The model under review builds one solid part; all positions refer to its coordinate system, in mm. A direction names the side the tool comes from. Coordinates: 2 decimals unless noted, no trailing zeros. Write each loop counter-clockwise with the first axis right and the second up, starting at its lowest first coordinate (ties: lowest second). Pieces come first, ordered by that corner, then holes. Notation, with made-up numbers: M 52,17.5 L 100,17.5 A26 cw 100,38.5 Z; hole C 49.25,11.25 d1. An arc over 180 degrees is marked long. Answer as CSV lines item,"result". Start each with the question number.
from build123d import *

# Parameters (mm, degrees)
EXTRUDE_1_DEPTH     = 40
CHAMFER_1_SIZE      = 3
CUT_EXTRUDE_1_DEPTH = 40
SKETCH_4_R          = 2.25
CUT_EXTRUDE_2_DEPTH = 40


with BuildPart() as part:
    # 草图2 → 凸台-拉伸1 (new body)
    with BuildSketch(Plane.XY):
        with BuildLine():
            Line((0, 0), (14.5, 0))
            ThreePointArc((14.5, 0), (16.621320344, 0.878679656), (17.5, 3))
            Line((17.5, 3), (17.5, 8))
            ThreePointArc((17.5, 8), (18.964466094, 11.535533906), (22.5, 13))
            Line((22.5, 13), (67.5, 13))
            ThreePointArc((67.5, 13), (71.035533906, 11.535533906), (72.5, 8))
            Line((72.5, 8), (72.5, 3))
            ThreePointArc((72.5, 3), (73.378679656, 0.878679656), (75.5, 0))
            Line((75.5, 0), (90, 0))
            Line((90, 0), (90, -2))
            Line((90, -2), (75.5, -2))
            ThreePointArc((75.5, -2), (71.964466094, -0.535533906), (70.5, 3))
            Line((70.5, 3), (70.5, 8))
            ThreePointArc((70.5, 8), (69.621320344, 10.121320344), (67.5, 11))
            Line((67.5, 11), (22.5, 11))
            ThreePointArc((22.5, 11), (20.378679656, 10.121320344), (19.5, 8))
            Line((19.5, 8), (19.5, 3))
            ThreePointArc((19.5, 3), (18.035533906, -0.535533906), (14.5, -2))
            Line((14.5, -2), (0, -2))
            Line((0, -2), (0, 0))
        make_face()
    extrude(amount=EXTRUDE_1_DEPTH)

    # 倒角1
    chamfer_1_edges = [part.edges().sort_by_distance(p)[0] for p in [
        (0, -1, 0),
        (90, -1, 0),
        (0, -1, 40),
        (90, -1, 40),
    ]]
    chamfer(chamfer_1_edges, length=CHAMFER_1_SIZE)

    # 草图3 → 切除-拉伸1 (cut)
    with BuildSketch(Plane(origin=(0, 0, 0), x_dir=(1, 0, 0), z_dir=(0, 1, 0))):
        with BuildLine():
            Line((4.25, -10), (4.25, -30))
            ThreePointArc((4.25, -30), (7.5, -33.25), (10.75, -30))
            Line((10.75, -30), (10.75, -10))
            ThreePointArc((10.75, -10), (7.5, -6.75), (4.25, -10))
        make_face()
        with BuildLine():
            ThreePointArc((85.75, -30), (82.5, -33.25), (79.25, -30))
            Line((79.25, -30), (79.25, -10))
            ThreePointArc((79.25, -10), (82.5, -6.75), (85.75, -10))
            Line((85.75, -10), (85.75, -30))
        make_face()
    extrude(amount=-CUT_EXTRUDE_1_DEPTH, mode=Mode.SUBTRACT)

    # 草图4 → 切除-拉伸2 (cut)
    with BuildSketch(Plane(origin=(0, 13, 0), x_dir=(1, 0, 0), z_dir=(0, 1, 0))):
        with Locations(Location((34.5, -18.5, 0), (0, 0, 270))):
            Circle(SKETCH_4_R)
        with Locations(Location((27, -20, 0), (0, 0, 270))):
            Circle(SKETCH_4_R)
        with Locations(Location((55.5, -18.5, 0), (0, 0, 270))):
            Circle(SKETCH_4_R)
        with Locations(Location((63, -20, 0), (0, 0, 270))):
            Circle(SKETCH_4_R)
        with Locations(Location((27, -5, 0), (0, 0, 270))):
            Circle(SKETCH_4_R)
        with Locations(Location((63, -5, 0), (0, 0, 270))):
            Circle(SKETCH_4_R)
    extrude(amount=-CUT_EXTRUDE_2_DEPTH, mode=Mode.SUBTRACT)


solid = part.part
1) Mouldability with a two-part tool opening along Z and no side actions: class faces 4 (the cylindrical face through (72, -0.57, 19.72)), 5 (the flat face through (45, 12, 40)), 6 (the cylindrical face through (82.57, -0.99, 33.25)) as +Z half, -Z half, draft (parallel to the pull), parting line (faces both ways), or undercut.
2) Take a section at A-A on x = 34.5. Give the boundary of the cut face in (y, z), and give its area (3 significant figures).
3) Clearance check with flat-ended pins moving along their axes: pin 1 Ø2 at (y, z) = (10.5, 24.5) entering from -X; pin 2 Ø5 at (x, z) = (63, 20) entering from -Y; pin 3 Ø5 at (x, y) = (38.5, 10.5) entering from +Z; pin 4 Ø5.5 at (y, z) = (5.5, 28) entering from +X. State where each tip first meets the part, or that it passes through.
4) Take a section at C-C on x = 63. Give the boundary of the cut face in (y, z), and give its area (3 significant figures).
5) Tool access review of faces 1 (the cylindrical face through (20.4, 10.14, 19.72)), 2 (the flat face through (72.5, 6, 20)), 3 (the cylindrical face through (7.57, -0.99, 6.75)): name each direction out of +Z, -Z, +X, -X, +Y, -Y from which nothing blocks a thin tool from reaching the whole face with its end or side.
6) To check wall thickness, follow line 1 (X direction, y = 11.7, z = 5); line 2 (X direction, y = 12.3, z = 5); line 3 (X direction, y = 6, z = 33). State the ranges of each line that lie inside material, in increasing order. Write a range as [from, to].
7) Take a section at D-D on x = 82.5. Give the boundary of the cut face in (y, z).
8) Take a section at B-B on z = 12. Give the boundary of the cut face in (x, y).
Results:
1,face 4,"draft"
1,face 5,"+Z half"
1,face 6,"undercut"
2,outline,"M 11,0 L 13,0 L 13,16.25 L 11,16.25 Z; M 11,20.75 L 13,20.75 L 13,40 L 11,40 Z"
2,area,"71.0 mm²"
3,pin 1,"stops at x = 17.73"
3,pin 2,"stops at y = 11"
3,pin 3,"stops at z = 40"
3,pin 4,"stops at x = 72.51"
4,outline,"M 11,0 L 13,0 L 13,2.75 L 11,2.75 Z; M 11,7.25 L 13,7.25 L 13,17.75 L 11,17.75 Z; M 11,22.25 L 13,22.25 L 13,40 L 11,40 Z"
4,area,"62.0 mm²"
5,face 1,"+Z, -Z, -Y"
5,face 2,"+Z, -Z, +X, +Y"
5,face 3,"+Y, -Y"
6,line 1,"x = [19.14, 24.75], [29.25, 60.75], [65.25, 70.86]"
6,line 2,"x = [19.95, 24.75], [29.25, 60.75], [65.25, 70.05]"
6,line 3,"x = [17.5, 19.5], [70.5, 72.5]"
7,outline,"M -2,0 L 0,0 L 0,6.75 L -2,6.75 Z; M -2,33.25 L 0,33.25 L 0,40 L -2,40 Z"
8,outline,"M 0,-2 L 4.25,-2 L 4.25,0 L 0,0 Z; M 10.75,-2 L 14.5,-2 A5 ccw 19.5,3 L 19.5,8 A3 cw 22.5,11 L 67.5,11 A3 cw 70.5,8 L 70.5,3 A5 ccw 75.5,-2 L 79.25,-2 L 79.25,0 L 75.5,0 A3 cw 72.5,3 L 72.5,8 A5 ccw 67.5,13 L 22.5,13 A5 ccw 17.5,8 L 17.5,3 A3 cw 14.5,0 L 10.75,0 Z; M 85.75,-2 L 90,-2 L 90,0 L 85.75,0 Z"
